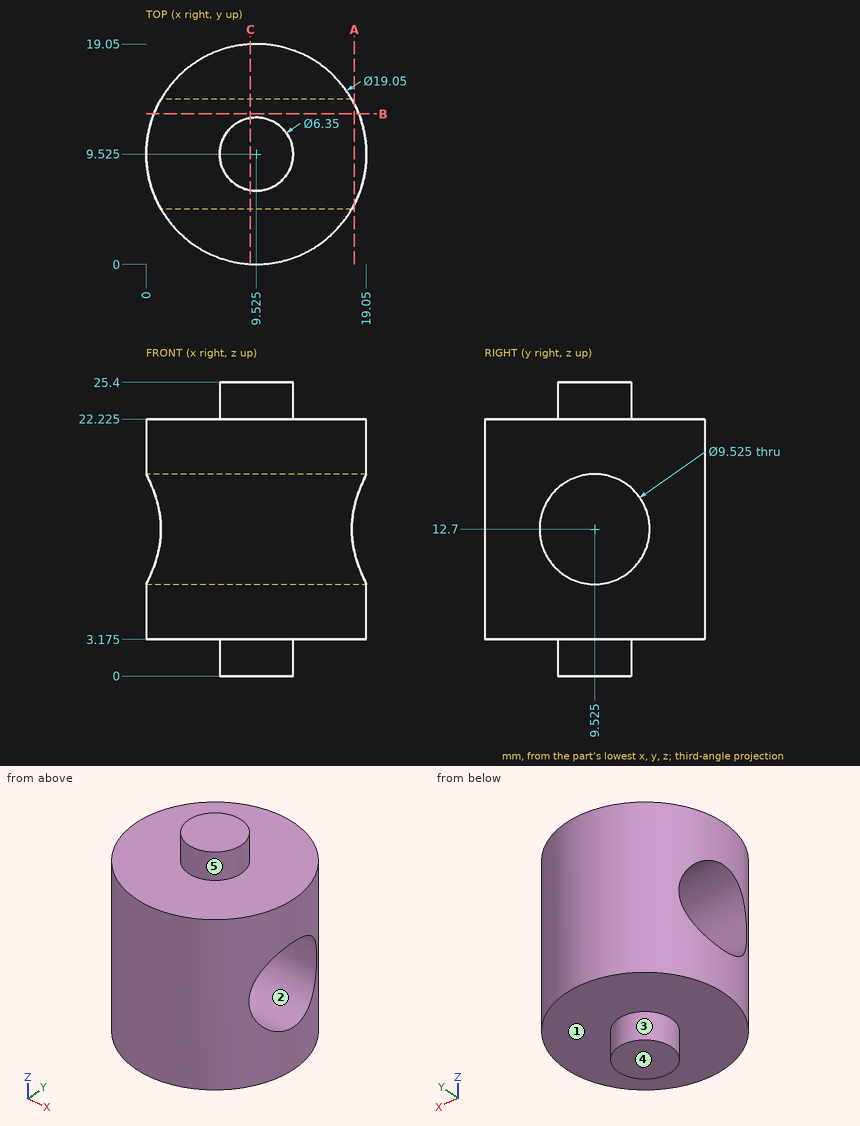
The figure shows three views and two pictorial views of one solid part (mm, origin at its lowest corner). Answer the questions. A direction names the side the tool comes from. Round coordinates to 2 decimals unless told otherwise and drop trailing zeros. Order: outer loops, then holes, each group sorted by start corner. A loop starts at its lowest first (then second) coordinate and runs counter-clockwise, first axis right, second up.
Q1. Find the intervals of material crossed by line 1 along Z through (x, y) = (2.25, 15) (3 decimals); line 2 along Y through (x, z) = (12.25, 16.5); line 3 along Y through (x, z) = (13.25, 12.7), in increasing order.
Solution:
line 1: z = 3.175 to 22.225
line 2: y = 0.4 to 6.65, 12.4 to 18.65
line 3: y = 0.76 to 4.76, 14.29 to 18.29
Q2. The mould has two halves that part along Y. Classify the marked faces 1, 2 and 3: pulls with the +Y half, pulls with the -Y half, needs draft (parallel to the pull), parting line crosses it, or undercut.
Solution:
face 1: needs draft
face 2: undercut
face 3: parting line crosses it
Q3. A cutting plane is placed at A-A, the plane x = 18. Determine the outline of the cut face in (y, z) (1 decimal), then the cut area to 3 significant figures.
Solution:
outline: (5.2, 3.2) - (13.9, 3.2) - (13.9, 10.8) arc R4.8 cw to (5.2, 10.8) - close; (5.2, 14.6) arc R4.8 cw to (13.9, 14.6) - (13.9, 22.2) - (5.2, 22.2) - close
area: 96.6 mm2
Q4. A cutting plane is placed at C-C, the plane x = 9. Determine the outline of the cut face in (y, z) (1 decimal).
Solution:
outline: (0, 3.2) - (6.4, 3.2) - (6.4, 0) - (12.7, 0) - (12.7, 3.2) - (19, 3.2) - (19, 22.2) - (12.7, 22.2) - (12.7, 25.4) - (6.4, 25.4) - (6.4, 22.2) - (0, 22.2) - close; hole circle Ø9.5 at (9.5, 12.7)
Q5. Given pin 1 Ø1.5 at (y, z) = (3.5, 11) entering from -X; pin 2 Ø4 at (y, z) = (8.5, 5.5) entering from +X; pin 3 Ø1.5 at (y, z) = (6.5, 22) entering from -X; pin 4 Ø7.5 at (y, z) = (9.525, 12.7) entering from -X, each flat-ended and moving along its own axis, determine where each tip first touches the part or whether it passes through.
Solution:
pin 1: stops at x = 1.59
pin 2: stops at x = 19.05
pin 3: stops at x = 0.28
pin 4: passes through
Q6. A cutting plane is placed at B-B, the plane y = 13. Determine the outline of the cut face in (x, z) (3 decimals).
Solution:
outline: (0.657, 3.175) - (18.393, 3.175) - (18.393, 9.443) - (0.657, 9.443) - close; (0.657, 15.957) - (18.393, 15.957) - (18.393, 22.225) - (0.657, 22.225) - close
Q7. A tool of negligible diameter and unlimited length cuts with its end or side. For the marked faces 4 and 5, from which of +Z, -Z, +X, -X, +Y, -Y can it reach the whole face along a straight path? Write none if from no direction.
Solution:
face 4: -Z, +X, -X, +Y, -Y
face 5: +Z
